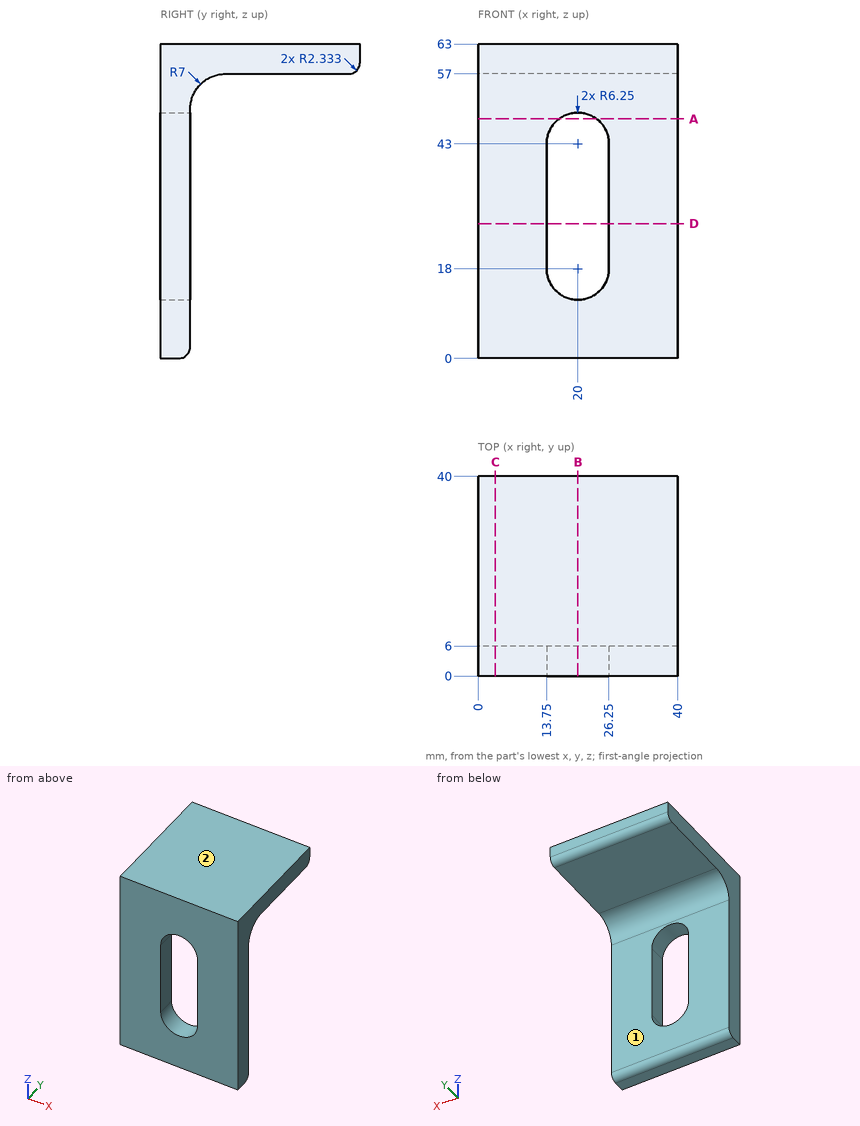
The drawing under review shows one solid part. Ordinate dimensions are in mm from its lowest x, y, z. A direction names the side the tool comes from. Give positions to 0.01 mm unless a question says otherwise; leave off trailing zeros. Loops run counter-clockwise (first coordinate to the right, second up) from the corner with the lowest first, then second, coordinate; pieces in that order, holes last. Notation, with made-up numbers: M 21,20 L 74,20 A13 cw 74,26 Z; hole C 63.25,-2.5 d5. An arc over 180 degrees is marked long. One line per item, written item: value. Start each with the question number.
Q1. Machinability: for the marked faces 1 and 2, which of the approach directions +Z, -Z, +X, -X, +Y, -Y give a long, thin tool a straight path to every point of the face, cutting with its end or side? Answer none if there is none.
Q2. Add section D-D (z = 27). Give the boundary of the cut face in (x, y).
Q3. For L1, parallel to Z at x = 12, y = 15; L2, parallel to Y at x = 8, z = 9.5; L3, parallel to Z at x = 17, y = 3, list the stretches that pass through material, from the lowest coordinate up.
Q4. Add section B-B (x = 20). Give the boundary of the cut face in (y, z), and give its area (3 significant figures).
Q5. Add section C-C (x = 3.5). Give the boundary of the cut face in (y, z).
Q6. Add section A-A (z = 48). Give the boundary of the cut face in (x, y).
Q7. Clearance check with flat-ended pins moving along their axes: pin 1 Ø2 at (x, y) = (23, 10) entering from -Z (1 decimal); pin 2 Ø3 at (x, z) = (27.5, 28) entering from +Y; pin 3 Ø12 at (x, z) = (26.5, 33.5) entering from -Y; pin 4 Ø4 at (x, z) = (7.5, 52) entering from +Y (1 decimal). State where each tip first meets the part, or that it passes through.
Reply:
1. face 1: -Z, +X, -X, +Y
1. face 2: +Z, +X, -X, +Y, -Y
2. outline: M 0,0 L 13.75,0 L 13.75,6 L 0,6 Z; M 26.25,0 L 40,0 L 40,6 L 26.25,6 Z
3. L1: 57 to 63
3. L2: 0 to 6
3. L3: 0 to 12.52, 48.48 to 63
4. outline: M 0,0 L 3.67,0 A2.33 ccw 6,2.33 L 6,11.75 L 0,11.75 Z; M 0,49.25 L 6,49.25 L 6,50 A7 cw 13,57 L 37.67,57 A2.33 ccw 40,59.33 L 40,63 L 0,63 Z
4. area: 365 mm²
5. outline: M 0,0 L 3.67,0 A2.33 ccw 6,2.33 L 6,50 A7 cw 13,57 L 37.67,57 A2.33 ccw 40,59.33 L 40,63 L 0,63 Z
6. outline: M 0,0 L 16.25,0 L 16.25,6 L 0,6 Z; M 23.75,0 L 40,0 L 40,6 L 23.75,6 Z
7. pin 1: z = 55.7
7. pin 2: y = 6
7. pin 3: y = 0
7. pin 4: y = 7.3
